Geometry check sheet. Reference: the model listing, model coordinates, mm. Face numbers are marked on the shaded views. A direction names the side the tool comes from. Round coordinates to 2 decimals unless told otherwise and drop trailing zeros. Order: outer loops, then holes, each group sorted by start corner. A loop starts at its lowest first (then second) coordinate and runs counter-clockwise, first axis right, second up.
(1) Release check for a two-part mould opening along Y. For the marked faces 4, 5, 6 and 7 record: +Y half, -Y half, draft (parallel to the pull), parting line (faces both ways), or undercut.
(2) Sectioned sample at B-B (x = 12.5). Record the boundary of the cut face in (y, z), plus the area to 3 significant figures.
(3) Sectioned sample at C-C (y = -18). Record the boundary of the cut face in (x, z), plus the area to 3 significant figures.
(4) Material ranges on line 1 along Y through (x, z) = (12.5, -19.5); line 2 along Y through (x, z) = (-12.5, -17.5); line 3 along Z through (x, y) = (-32, -34), recorded low to high.
(5) Set-up check for the marked faces 1, 2 and 3: record each of +Z, -Z, +X, -X, +Y, -Y from which the full face is reachable in a straight line by a thin tool's end or side.
(6) Sectioned sample at A-A (y = -42). Record the boundary of the cut face in (x, z), plus the area to 3 significant figures.
(7) Sectioned sample at D-D (x = -1). Record the boundary of the cut face in (y, z).
(8) Go/stop test with flat-tipped pins: pin 1 (1 mm diameter, centred on x = -18, y = 28, fed in from +Z); pin 2 (1.4 mm diameter, centred on y = 11, z = 36, fed in from -X); pin 3 (5 mm diameter, centred on x = 16.5, z = 19.5, fed in from +Y). Record where each tip stops, or that it passes through.
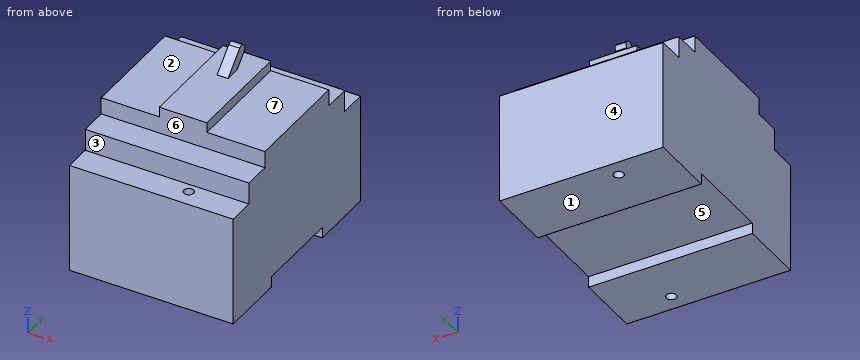
from build123d import *

# Parameters (mm, degrees)
SKETCH1_W                  = 74.7
SKETCH1_H                  = 99.6
BOSS_EXTRUDE1_DEPTH        = 33.85
F_4_5_4_5_DIAMETER_HOLE1_D = 4.5
SKETCH4_W                  = 74.7
SKETCH4_H                  = 12.3
CUT_EXTRUDE1_DEPTH         = 17.7
SKETCH5_W                  = 74.7
SKETCH5_H                  = 12.5
CUT_EXTRUDE2_DEPTH         = 7.7
SKETCH6_W                  = 21.7
SKETCH6_H                  = 50
BOSS_EXTRUDE2_DEPTH        = 4.6
SKETCH7_W                  = 5
SKETCH7_H                  = 40
CUT_EXTRUDE3_DEPTH         = 118.6
BOSS_EXTRUDE3_DEPTH        = 2.5
FILLET1_R                  = 2


with BuildPart() as part:
    # Sketch1 → Boss-Extrude1 (new, symmetric)
    with BuildSketch(Plane.XY):
        Rectangle(SKETCH1_W, SKETCH1_H)
    extrude(amount=BOSS_EXTRUDE1_DEPTH, both=True)

    # Ø4.5 (4.5) Diameter Hole1 (through all)
    with Locations(Plane.XY.offset(33.85)):
        with Locations((-12.5, 42), (12.5, -42)):
            Hole(F_4_5_4_5_DIAMETER_HOLE1_D / 2)

    # Sketch4 → Cut-Extrude1 (cut)
    with BuildSketch(Plane.XY.offset(33.85)):
        with Locations((0, 43.65)):
            Rectangle(SKETCH4_W, SKETCH4_H)
        with Locations((0, -43.65)):
            Rectangle(SKETCH4_W, SKETCH4_H)
    extrude(amount=-CUT_EXTRUDE1_DEPTH, mode=Mode.SUBTRACT)

    # Sketch5 → Cut-Extrude2 (cut)
    with BuildSketch(Plane.XY.offset(33.85)):
        with Locations((0, -31.25)):
            Rectangle(SKETCH5_W, SKETCH5_H)
        with Locations((0, 31.25)):
            Rectangle(SKETCH5_W, SKETCH5_H)
    extrude(amount=-CUT_EXTRUDE2_DEPTH, mode=Mode.SUBTRACT)

    # Sketch6 → Boss-Extrude2 (add)
    with BuildSketch(Plane.XY.offset(33.85)):
        Rectangle(SKETCH6_W, SKETCH6_H)
    extrude(amount=BOSS_EXTRUDE2_DEPTH)

    # Sketch7 → Cut-Extrude3 (cut)
    with BuildSketch(Plane(origin=(37.35, 0, 0), x_dir=(0, 0, -1), z_dir=(1, 0, 0))):
        with Locations((31.35, 0)):
            Rectangle(SKETCH7_W, SKETCH7_H)
    extrude(amount=-CUT_EXTRUDE3_DEPTH, mode=Mode.SUBTRACT)

    # Sketch8 → Boss-Extrude3 (add, symmetric)
    with BuildSketch(Plane(origin=(0, 0, 0), x_dir=(0, 0, -1), z_dir=(1, 0, 0))):
        Polygon((-38.45, 13), (-45.45, 20), (-48.985533906, 16.464466094), (-38.45, 5.928932188), align=None)
    extrude(amount=BOSS_EXTRUDE3_DEPTH, both=True)

    # Fillet1
    fillet1_edges = [part.edges().sort_by_distance(p)[0] for p in [
        (0, 20, 45.45),
        (0, 16.464466094, 48.985533906),
    ]]
    fillet(fillet1_edges, radius=FILLET1_R)


solid = part.part
Answer below:
1. face 4: +Y half
1. face 5: undercut
1. face 6: -Y half
1. face 7: draft
2. outline: (-49.8, -33.85) - (-44.25, -33.85) - (-44.25, 16.15) - (-49.8, 16.15) - close; (-39.75, -33.85) - (-20, -33.85) - (-20, -28.85) - (20, -28.85) - (20, -33.85) - (49.8, -33.85) - (49.8, 16.15) - (37.5, 16.15) - (37.5, 26.15) - (25, 26.15) - (25, 33.85) - (-25, 33.85) - (-25, 26.15) - (-37.5, 26.15) - (-37.5, 16.15) - (-39.75, 16.15) - close
2. area: 5,690 mm2
3. outline: (-37.35, -28.85) - (37.35, -28.85) - (37.35, 33.85) - (10.85, 33.85) - (10.85, 38.45) - (-10.85, 38.45) - (-10.85, 33.85) - (-37.35, 33.85) - close
3. area: 4,780 mm2
4. line 1: y = -49.8 to -44.25, -39.75 to 49.8
4. line 2: y = -49.8 to 39.75, 44.25 to 49.8
4. line 3: z = -33.85 to 26.15
5. face 1: -Z, +X, -X, +Y, -Y
5. face 2: +Z, -X, +Y, -Y
5. face 3: +Z, +X, -X, -Y
6. outline: (-37.35, -33.85) - (10.25, -33.85) - (10.25, 16.15) - (-37.35, 16.15) - close; (14.75, -33.85) - (37.35, -33.85) - (37.35, 16.15) - (14.75, 16.15) - close
6. area: 3,510 mm2
7. outline: (-49.8, -33.85) - (-20, -33.85) - (-20, -28.85) - (20, -28.85) - (20, -33.85) - (49.8, -33.85) - (49.8, 16.15) - (37.5, 16.15) - (37.5, 26.15) - (25, 26.15) - (25, 38.45) - (13, 38.45) - (18.59, 44.04) arc R2 ccw to (18.59, 46.86) - (17.88, 47.57) arc R2 ccw to (15.05, 47.57) - (5.93, 38.45) - (-25, 38.45) - (-25, 26.15) - (-37.5, 26.15) - (-37.5, 16.15) - (-49.8, 16.15) - close
8. pin 1: stops at z = 26.15
8. pin 2: stops at x = -10.85
8. pin 3: stops at y = 37.5
